For this review, take the finished solid that the model builds, in its own axes (mm). Face numbers are marked on the shaded views. A direction names the side the tool comes from. Coordinates: 2 decimals unless noted, no trailing zeros. Write each loop counter-clockwise with the first axis right and the second up, starting at its lowest first coordinate (ties: lowest second). Pieces come first, ordered by that corner, then holes. Notation, with made-up numbers: M -37,62.25 L -32,62.25 A22 ccw -32,93.25 Z; hole C 56,29.25 d9. An arc over 180 degrees is marked long. Return JSON: item names as keys, results as strings.
```python
from build123d import *

# Parameters (mm, degrees)
HOLE_WIZARD_M6_1_D           = 6.6
HOLE_WIZARD_M6_1_CBORE_D     = 11
HOLE_WIZARD_M6_1_CBORE_DEPTH = 6.4
SKETCH_4_R                   = 16
CUT_EXTRUDE_1_DEPTH          = 67.543219038
EXTRUDE_1_DEPTH              = 10
SKETCH_6_W                   = 38
SKETCH_6_H                   = 16
CUT_EXTRUDE_2_DEPTH          = 10
CUT_EXTRUDE_3_DEPTH          = 74.810568349
CUT_EXTRUDE_3_DEPTH_BACK     = 74.810568349
SKETCH_7_R                   = 2
SKETCH_9_R                   = 20
CUT_EXTRUDE_5_DEPTH          = 34
SKETCH_10_W                  = 100
SKETCH_10_H                  = 16
CUT_EXTRUDE_6_DEPTH          = 12
HOLE_WIZARD_M4_1_D           = 3.3


with BuildPart() as part:
    # 草图1 → 旋转1 (revolve)
    with BuildSketch(Plane.XY, mode=Mode.PRIVATE) as revolve_1_sk:
        Polygon((0, 46), (34, 46), (34, 36), (18.4, 36), (18.4, 26), (17.492059993, 0), (0, 0), align=None)
    revolve(revolve_1_sk.sketch.rotate(Axis((0, 0, 0), (0, 1, 0)), 90), axis=Axis((0, 0, 0), (0, 1, 0)))

    # M6 六角凹头螺钉的柱形沉头孔1 (through all)
    with Locations(Plane(origin=(0, 46, 0), x_dir=(1, 0, 0), z_dir=(0, 1, 0))):
        with Locations((0, 25), (0, -25)):
            CounterBoreHole(HOLE_WIZARD_M6_1_D / 2, HOLE_WIZARD_M6_1_CBORE_D / 2, HOLE_WIZARD_M6_1_CBORE_DEPTH)

    # 草图4 → 切除-拉伸1 (cut, through all)
    with BuildSketch(Plane(origin=(0, 46, 0), x_dir=(1, 0, 0), z_dir=(0, 1, 0))):
        with Locations(Location((0, 0, 0), (0, 0, 270))):
            Circle(SKETCH_4_R)
    extrude(amount=-CUT_EXTRUDE_1_DEPTH, mode=Mode.SUBTRACT)

    # 草图5 → 凸台-拉伸1 (add)
    with BuildSketch(Plane(origin=(0, 46, 0), x_dir=(1, 0, 0), z_dir=(0, 1, 0))):
        with BuildLine():
            Line((33.045423284, -8), (13.856406461, -8))
            ThreePointArc((13.856406461, -8), (16, 0), (13.856406461, 8))
            Line((13.856406461, 8), (33.045423284, 8))
            ThreePointArc((33.045423284, 8), (34, 0), (33.045423284, -8))
        make_face()
        with BuildLine():
            Line((-33.045423284, 8), (-13.856406461, 8))
            ThreePointArc((-13.856406461, 8), (-16, 0), (-13.856406461, -8))
            Line((-13.856406461, -8), (-33.045423284, -8))
            ThreePointArc((-33.045423284, -8), (-34, 0), (-33.045423284, 8))
        make_face()
    extrude(amount=EXTRUDE_1_DEPTH)

    # 草图6 → 切除-拉伸2 (cut)
    with BuildSketch(Plane(origin=(0, 56, 0), x_dir=(1, 0, 0), z_dir=(0, 1, 0))):
        Rectangle(SKETCH_6_W, SKETCH_6_H)
    extrude(amount=-CUT_EXTRUDE_2_DEPTH, mode=Mode.SUBTRACT)

    # 草图7 → 切除-拉伸3 (cut, two sides: drawn at the far end of the back side and taken through both)
    with BuildSketch(Plane(origin=(0, 0, 0), x_dir=(0, 0, -1), z_dir=(1, 0, 0)).offset(-CUT_EXTRUDE_3_DEPTH_BACK)):
        with Locations((0, 50)):
            Circle(SKETCH_7_R)
    extrude(amount=CUT_EXTRUDE_3_DEPTH + CUT_EXTRUDE_3_DEPTH_BACK, mode=Mode.SUBTRACT)

    # 草图9 → 切除-拉伸5 (cut)
    with BuildSketch(Plane.XZ):
        Circle(SKETCH_9_R)
    extrude(amount=-CUT_EXTRUDE_5_DEPTH, mode=Mode.SUBTRACT)

    # 草图10 → 切除-拉伸6 (cut)
    with BuildSketch(Plane(origin=(0, 56, 0), x_dir=(1, 0, 0), z_dir=(0, 1, 0))):
        Rectangle(SKETCH_10_W, SKETCH_10_H)
    extrude(amount=-CUT_EXTRUDE_6_DEPTH, mode=Mode.SUBTRACT)

    # M4 螺纹孔1 (through all)
    with Locations(Plane(origin=(0, 46, 0), x_dir=(1, 0, 0), z_dir=(0, 1, 0))):
        with Locations((-25, 0), (25, 0)):
            Hole(HOLE_WIZARD_M4_1_D / 2)


solid = part.part
```
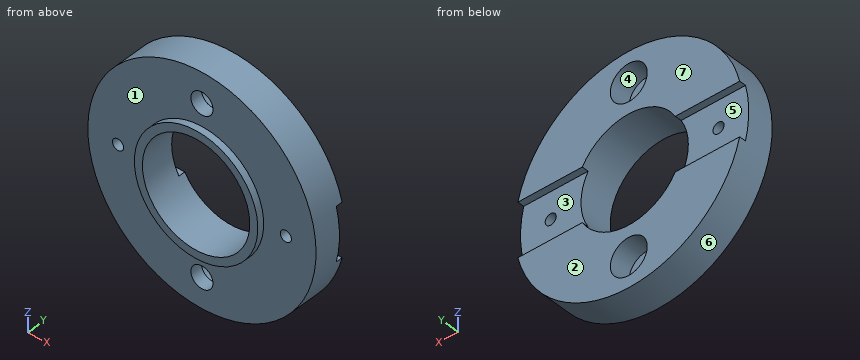
1. For the marked faces 1, 2, 3 and 4, list the 3-axis set-ups (+Z, -Z, +X, -X, +Y, -Y) from which the entire face can be reached by the end or side of a thin tool; tool diameter is ignored.
Checks:
{"face 1": "-Y", "face 2": "+Z, -Z, +X, -X, +Y", "face 3": "+X, -X, +Y", "face 4": "+Y"}
2. We need section C-C (x = -11). State the section outline as (y, z) points.
Checks:
{"outline": "M 34,-14.75 L 36,-14.75 L 36,-32.17 L 46,-32.17 L 46,-11.62 L 34,-11.62 Z; M 34,11.62 L 46,11.62 L 46,32.17 L 36,32.17 L 36,14.75 L 34,14.75 Z"}
3. Draft analysis for pull direction Z (two halves, no side actions). For the marked faces 5, 6 and 7, state which applies: +Z half, -Z half, draft (parallel to the pull), parting line (faces both ways), or undercut.
Checks:
{"face 5": "undercut", "face 6": "parting line", "face 7": "draft"}
4. We need section D-D (y = 41). State the section outline as (x, z) points.
Checks:
{"outline": "C 0,0 d68; hole C -25,0 d3.3; hole C 0,0 d32; hole C 0,-25 d11; hole C 0,25 d11; hole C 25,0 d3.3"}
5. Clearance check with flat-ended pins moving along their axes: pin 1 Ø2 at (x, y) = (28, 45.5) entering from +Z; pin 2 Ø4.5 at (x, z) = (25, 0) entering from -Y; pin 3 Ø1 at (x, z) = (24, -3) entering from +Y. State where each tip first meets the part, or that it passes through.
Checks:
{"pin 1": "z = 20.66", "pin 2": "y = 36", "pin 3": "y = 44"}
6. We need section B-B (z = -3). State the section outline as (x, y) points.
Checks:
{"outline": "M -33.87,36 L -18.15,36 L -18.15,34 L -15.72,34 L -15.72,44 L -33.87,44 Z; M 15.72,34 L 18.15,34 L 18.15,36 L 33.87,36 L 33.87,44 L 15.72,44 Z"}
7. Wall thickness on L1, parallel to X at y = 41, z = -3; L2, parallel to Y at x = 7, z = 24; L3, parallel to Y at x = 19.5, z = 5.5: over which ranges is each line inside the solid? List them lowest first. Write a range as from..to.
Checks:
{"L1": "-33.87..-15.72, 15.72..33.87", "L2": "36..46", "L3": "36..44"}
8. We need section A-A (y = 45). State the section outline as (x, z) points, plus the area to 3 significant figures.
Checks:
{"outline": "M -33.05,-8 A34 ccw 33.05,-8 L 13.86,-8 A16 cw -13.86,-8 Z; M -33.05,8 L -13.86,8 A16 cw 13.86,8 L 33.05,8 A34 ccw Z; hole C 0,-25 d11; hole C 0,25 d11", "area": "2,050 mm2"}
